Work out the finished part from the listing and answer in its coordinate system (mm). Round coordinates to 2 decimals unless told otherwise and drop trailing zeros. Loops run counter-clockwise (first coordinate to the right, second up) from the corner with the lowest first, then second, coordinate; pieces in that order, holes last. Notation, with made-up numbers: (-9, 40) -> (-5, 40) arc R25 ccw to (-5, 59) -> close; hole circle Ø7 at (5.5, -12). An arc over 180 degrees is marked (long way). Use one line per item in the form item = value.
```python
from build123d import *

# Parameters (mm, degrees)
SKETCH1_R           = 55
SKETCH1_R_2         = 50
BOSS_EXTRUDE1_DEPTH = 11.75
CHAMFER1_SIZE       = 1
CHAMFER2_SIZE       = 2


with BuildPart() as part:
    # Sketch1 → Boss-Extrude1 (new body)
    with BuildSketch(Plane(origin=(0, 0, 0), x_dir=(1, 0, 0), z_dir=(0, 1, 0))):
        with Locations(Location((0, 0, 0), (0, 0, 270))):
            Circle(SKETCH1_R)
        with Locations(Location((0, 0, 0), (0, 0, 270))):
            Circle(SKETCH1_R_2, mode=Mode.SUBTRACT)
    extrude(amount=BOSS_EXTRUDE1_DEPTH)

    # Chamfer1
    chamfer1_edges = [part.edges().sort_by_distance(p)[0] for p in [
        (0, 0, -55),
        (0, 11.75, -55),
    ]]
    chamfer(chamfer1_edges, length=CHAMFER1_SIZE)

    # Chamfer2
    chamfer2_edges = [part.edges().sort_by_distance(p)[0] for p in [
        (0, 0, -50),
        (0, 11.75, -50),
    ]]
    chamfer(chamfer2_edges, length=CHAMFER2_SIZE)


solid = part.part
```
(1) For a pull along Z with two mould halves and no side action, classify faces 1 (the flat face through (44, 11.75, -28)), 2 (the cylindrical face through (-48.794, 5.807, 25.379)), 3 (the conical face through (34, 10, -37)) as +Z half, -Z half, draft (parallel to the pull), parting line (faces both ways), or undercut.
Completed:
face_1 = draft
face_2 = parting line
face_3 = undercut
(2) Consider L1, parallel to X at y = 8, z = 0; L2, parallel to Z at x = 2, y = 9.25; L3, parallel to X at y = 9.5, z = -41.5. Determine where each line is inside the solid, lowest interval first.
Completed:
L1 = -55 to -50, 50 to 55
L2 = -54.96 to -49.96, 49.96 to 54.96
L3 = -36.09 to -27.89, 27.89 to 36.09
(3) Find section A-A, the plane x = 0. Write down the section's boundary in (y, z).
Completed:
outline = (0, -54) -> (1, -55) -> (10.75, -55) -> (11.75, -54) -> (11.75, -52) -> (9.75, -50) -> (2, -50) -> (0, -52) -> close; (0, 52) -> (2, 50) -> (9.75, 50) -> (11.75, 52) -> (11.75, 54) -> (10.75, 55) -> (1, 55) -> (0, 54) -> close
(4) Find section B-B, the plane z = 0. Write down the section's boundary in (x, y).
Completed:
outline = (-55, 1) -> (-54, 0) -> (-52, 0) -> (-50, 2) -> (-50, 9.75) -> (-52, 11.75) -> (-54, 11.75) -> (-55, 10.75) -> close; (50, 2) -> (52, 0) -> (54, 0) -> (55, 1) -> (55, 10.75) -> (54, 11.75) -> (52, 11.75) -> (50, 9.75) -> close
(5) Find section C-C, the plane y = 7. Write down the section's boundary in (x, z), then the cut area to 3 significant figures.
Completed:
outline = circle Ø110 at (0, 0); hole circle Ø100 at (0, 0)
area = 1,650 mm2
(6) Given P1, Ø3, axis at x = 25.5, y = 10, coming from the +Z side; P2, Ø1.5, axis at x = -41, y = 3, coming from the +Z side; P3, Ø6, axis at y = 7.5, z = 10, coming from the -X side, each flat-ended and moving along its own axis, determine where each tip first touches the part or whether it passes through.
Completed:
P1 = 49.49
P2 = 37.48
P3 = -54.55
